Part model, mm, in its own coordinate system. Give positions to 0.01 mm unless a question says otherwise; leave off trailing zeros. Order: outer loops, then holes, each group sorted by start corner. A loop starts at its lowest first (then second) coordinate and runs counter-clockwise, first axis right, second up. Notation, with made-up numbers: M 55,35 L 73,35 A15 ccw 73,54 Z; hole C 38.5,73 d2. An arc over 180 degrees is marked long. Return JSON: item names as keys, results as strings.
from build123d import *

# Parameters (mm, degrees)
SKETCH_1_R               = 230
EXTRUDE_1_DEPTH          = 10
SKETCH_2_R               = 105
CUT_EXTRUDE_1_DEPTH      = 326.883414736
SKETCH_3_R               = 150
SKETCH_3_R_2             = 105
EXTRUDE_2_DEPTH          = 20
HOLE_WIZARD_M12_1_D      = 10.2
PATTERN_CIRCULAR_1_COUNT = 16
HOLE_WIZARD_M12_1_2_D    = 13.5


with BuildPart() as part:
    # 草图1 → 凸台-拉伸1 (new, symmetric)
    with BuildSketch(Plane.XY):
        Circle(SKETCH_1_R)
    extrude(amount=EXTRUDE_1_DEPTH, both=True)

    # 草图2 → 切除-拉伸1 (cut, through all)
    with BuildSketch(Plane(origin=(0, 0, -10), x_dir=(-1, 0, 0), z_dir=(0, 0, -1))):
        Circle(SKETCH_2_R)
    extrude(amount=-CUT_EXTRUDE_1_DEPTH, mode=Mode.SUBTRACT)

    # 草图3 → 凸台-拉伸2 (add)
    with BuildSketch(Plane.XY.offset(10)):
        Circle(SKETCH_3_R)
        with Locations(Location((0, 0, 0), (0, 0, 180))):
            Circle(SKETCH_3_R_2, mode=Mode.SUBTRACT)
    extrude(amount=EXTRUDE_2_DEPTH)

    # Hole Wizard M12 _1 (through all)
    with Locations(Plane.XY.offset(30)):
        with Locations((112.365701655, -42.118275031)):
            hole_wizard_m12_1 = Hole(HOLE_WIZARD_M12_1_D / 2)

    # 阵列(圆周)1: Hole Wizard M12 _1 ×16 about axis
    pattern_circular_1_axis = Axis((0, 0, 0), (0, 0, 1))
    for i in range(1, PATTERN_CIRCULAR_1_COUNT):
        add(hole_wizard_m12_1.rotate(pattern_circular_1_axis, i * 360 / PATTERN_CIRCULAR_1_COUNT), mode=Mode.SUBTRACT)

    # Hole Wizard M12 _1 2 (through all)
    with Locations(Plane.XY.offset(10)):
        with Locations((54.118704372, -171.719208219), (80.088559574, -161.251800671), (171.165878787, 87.858133743), (184.250138222, 55.395814741), (-171.165880115, -87.858134279), (-184.25013955, -55.395815276), (-80.649167813, 162.642677508), (-54.679312611, 173.110085056)):
            Hole(HOLE_WIZARD_M12_1_2_D / 2)


solid = part.part
Q1. Band-saw the part on B-B (x = -31). Give the cut face in (y, z).
Established:
{"outline": "M -227.9,-10 L -100.32,-10 L -100.32,30 L -146.76,30 L -146.76,10 L -227.9,10 Z; M 100.32,-10 L 227.9,-10 L 227.9,10 L 146.76,10 L 146.76,30 L 100.32,30 Z"}
Q2. Two-plate mould, pull along Y, no slides. Class faces 1 (the cylindrical face through (-49.86, -224.53, 0.14)), 2 (the cylindrical face through (-177.401, -90.443, -0.14)), 3 (the flat face through (31, 102, 30)): +Y half, -Y half, draft (parallel to the pull), parting line (faces both ways), or undercut.
Established:
{"face 1": "parting line", "face 2": "undercut", "face 3": "draft"}
Q3. Band-saw the part on A-A (z = 22.5). Give the number of separate pieces and of enclosed holes in the cut face, then the cut area to 3 significant figures.
Established:
{"separate pieces": "1", "enclosed holes": "17", "area": "34,700 mm²"}
Q4. Band-saw the part on D-D (y = 198). Give the cut face in (x, z), then the cut area to 3 significant figures.
Established:
{"outline": "M -117.03,-10 L 117.03,-10 L 117.03,10 L -117.03,10 Z", "area": "4,680 mm²"}
Q5. Pin check, flat tips, straight feed: pin 1 (5 mm diameter, centred on y = -179.5, z = 11.5, fed in from +X); pin 2 (6 mm diameter, centred on x = -42.12, y = -112.37, fed in from +Z); pin 3 (3 mm diameter, centred on y = -69.5, z = 16, fed in from -X); pin 4 (17.5 mm diameter, centred on x = -80.65, y = 162.64, fed in from +Z). Stop position of each tip, or through.
Established:
{"pin 1": "stops at x = 146.27", "pin 2": "passes through", "pin 3": "stops at x = -133.7", "pin 4": "stops at z = 10"}
Q6. Probe line 1 along X through (y, z) = (-3, 20); line 2 along X through (y, z) = (60, -0.5); line 3 along Z through (x, y) = (176.5, 71.5). List the from-to ranges inside material, lowest first.
Established:
{"line 1": "x = -149.97 to -124.91, -114.95 to -104.96, 104.96 to 149.97", "line 2": "x = -222.04 to -86.17, 86.17 to 179.31, 189.19 to 222.04", "line 3": "z = -10 to 10"}
